Can you work these out from the model? Positions are in its coordinate system, mm. A direction names the side the tool comes from. Give positions to 0.01 mm unless a question says otherwise; leave off trailing zeros. Order: outer loops, then holes, each group sorted by start corner. A loop starts at its lowest first (then second) coordinate and runs counter-clockwise, first axis right, second up. Notation, with made-up numbers: M 47,60.25 L 97,60.25 A19 ccw 97,96.25 Z; hole C 16,-9.75 d11. An arc over 180 degrees is marked long. Answer as a JSON object with one key per item and string values.
```python
from build123d import *

# Parameters (mm, degrees)
BOSS_EXTRUDE1_DEPTH = 30
CUT_EXTRUDE1_DEPTH  = 25


with BuildPart() as part:
    # Sketch1 → Boss-Extrude1 (new body)
    with BuildSketch(Plane(origin=(0, 0, 0), x_dir=(1, 0, 0), z_dir=(0, 1, 0))):
        with BuildLine():
            Line((-220, 225), (220, 225))
            ThreePointArc((220, 225), (241.213203436, 216.213203436), (250, 195))
            Line((250, 195), (250, -195))
            ThreePointArc((250, -195), (241.213203436, -216.213203436), (220, -225))
            Line((220, -225), (-220, -225))
            ThreePointArc((-220, -225), (-241.213203436, -216.213203436), (-250, -195))
            Line((-250, -195), (-250, 195))
            ThreePointArc((-250, 195), (-241.213203436, 216.213203436), (-220, 225))
        make_face()
    extrude(amount=BOSS_EXTRUDE1_DEPTH)

    # Sketch2 → Cut-Extrude1 (cut)
    with BuildSketch(Plane(origin=(0, 30, 0), x_dir=(1, 0, 0), z_dir=(0, 1, 0))):
        with BuildLine():
            Line((-217, 222), (217, 222))
            ThreePointArc((217, 222), (238.213203436, 213.213203436), (247, 192))
            Line((247, 192), (247, -192))
            ThreePointArc((247, -192), (238.213203436, -213.213203436), (217, -222))
            Line((217, -222), (-217, -222))
            ThreePointArc((-217, -222), (-238.213203436, -213.213203436), (-247, -192))
            Line((-247, -192), (-247, 192))
            ThreePointArc((-247, 192), (-238.213203436, 213.213203436), (-217, 222))
        make_face()
    extrude(amount=-CUT_EXTRUDE1_DEPTH, mode=Mode.SUBTRACT)


solid = part.part
```
1) I want a section at A-A on y = 11.5. Write out the boundary of the cut face in (x, z).
Results found:
{"outline": "M -250,-195 A30 ccw -220,-225 L 220,-225 A30 ccw 250,-195 L 250,195 A30 ccw 220,225 L -220,225 A30 ccw -250,195 Z; hole M -247,-192 A30 ccw -217,-222 L 217,-222 A30 ccw 247,-192 L 247,192 A30 ccw 217,222 L -217,222 A30 ccw -247,192 Z"}
2) Thinking about a two-plate mould opening in X: for faces 1 (the face through (241.445, 14.79, 215.979)), 2 (the face through (237.979, 17.675, -213.445)), 3 (the face through (-250, 15, 3)), 4 (the face through (3, 0, -3)), which applies, pulls with the +X half, pulls with the -X half, needs draft (parallel to the pull), parting line crosses it, or undercut?
Results found:
{"face 1": "pulls with the +X half", "face 2": "undercut", "face 3": "pulls with the -X half", "face 4": "needs draft"}
3) I need wall thicknesses on L1, parallel to X at y = 22, z = -160.5; L2, parallel to Z at x = -19.5, y = 19.25; L3, parallel to Y at x = 198.5, z = 205. Which ranges of each line are inside material? Lowest first, please.
Results found:
{"L1": "x = -250 to -247, 247 to 250", "L2": "z = -225 to -222, 222 to 225", "L3": "y = 0 to 5"}
4) I want a section at C-C on z = -55. Write out the boundary of the cut face in (x, y).
Results found:
{"outline": "M -250,0 L 250,0 L 250,30 L 247,30 L 247,5 L -247,5 L -247,30 L -250,30 Z"}
5) I want a section at B-B on x = -165.5. Write out the boundary of the cut face in (y, z), and give its area (3 significant figures).
Results found:
{"outline": "M 0,-225 L 30,-225 L 30,-222 L 5,-222 L 5,222 L 30,222 L 30,225 L 0,225 Z", "area": "2,400 mm²"}
6) For faces 5 (the face through (238.445, 17.675, 212.979)), 6 (the face through (3, 15, 225)), which set-ups out of +Z, -Z, +X, -X, +Y, -Y let a thin tool reach every point of the face, with its end or its side?
Results found:
{"face 5": "+Y", "face 6": "+Z, +X, -X, +Y, -Y"}
7) I'm going to push a flat-ended pin straight in: pin 1 Ø6 at (x, z) = (141, 65.5) entering from +Y. Where does the tip first touch, or does it pass through?
Results found:
{"pin 1": "stops at y = 5"}
